For this review, use the dimensioned drawing (mm, ordinates from the lowest corner) and the shaded views. A direction names the side the tool comes from. Give positions to 0.01 mm unless a question says otherwise; leave off trailing zeros. Write each loop counter-clockwise with the first axis right and the second up, starting at its lowest first coordinate (ties: lowest second). Pieces come first, ordered by that corner, then holes. Notation, with made-up numbers: (21.25, 30.25) -> (75.25, 30.25) arc R23 ccw to (75.25, 62.25) -> close; hole circle Ø4 at (9, -34). An arc over 180 degrees is marked (long way). Return JSON: item names as keys, results as strings.
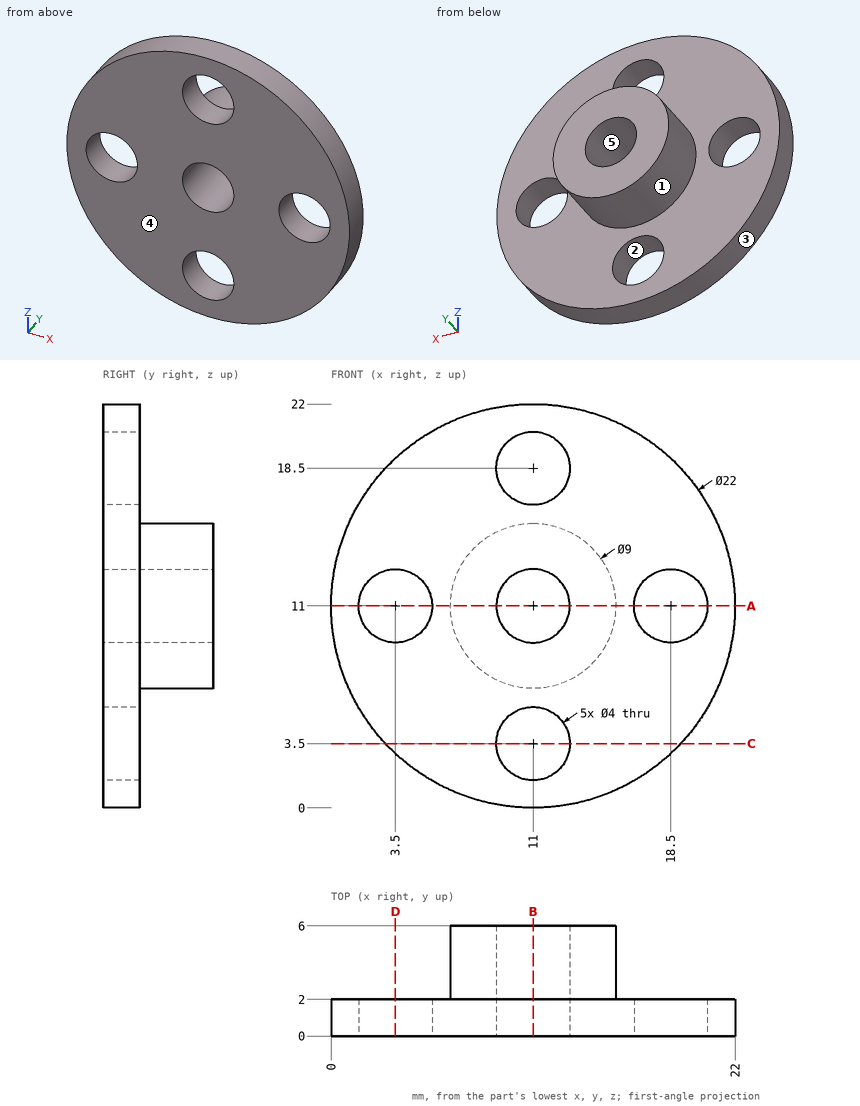
1. Add section C-C, the plane z = 3.5. State the section outline as (x, y) points.
Results found:
{"outline": "(2.95, 0) -> (9, 0) -> (9, 2) -> (2.95, 2) -> close; (13, 0) -> (19.05, 0) -> (19.05, 2) -> (13, 2) -> close"}
2. The part is to be moulded in two halves that separate along X. For the marked faces 3, 4 and 5, say which applies: +X half, -X half, draft (parallel to the pull), parting line (faces both ways), or undercut.
Results found:
{"face 3": "parting line", "face 4": "draft", "face 5": "undercut"}
3. For the marked faces 1 and 2, list the 3-axis set-ups (+Z, -Z, +X, -X, +Y, -Y) from which the entire face can be reached by the end or side of a thin tool; tool diameter is ignored.
Results found:
{"face 1": "+Y", "face 2": "+Y, -Y"}
4. Add section B-B, the plane x = 11. State the section outline as (y, z) points.
Results found:
{"outline": "(0, 0) -> (2, 0) -> (2, 1.5) -> (0, 1.5) -> close; (0, 5.5) -> (2, 5.5) -> (2, 6.5) -> (6, 6.5) -> (6, 9) -> (0, 9) -> close; (0, 13) -> (6, 13) -> (6, 15.5) -> (2, 15.5) -> (2, 16.5) -> (0, 16.5) -> close; (0, 20.5) -> (2, 20.5) -> (2, 22) -> (0, 22) -> close"}
5. Add section D-D, the plane x = 3.5. State the section outline as (y, z) points.
Results found:
{"outline": "(0, 2.95) -> (2, 2.95) -> (2, 9) -> (0, 9) -> close; (0, 13) -> (2, 13) -> (2, 19.05) -> (0, 19.05) -> close"}
6. Add section A-A, the plane z = 11. State the section outline as (x, y) points, plus the area to 3 significant figures.
Results found:
{"outline": "(0, 0) -> (1.5, 0) -> (1.5, 2) -> (0, 2) -> close; (5.5, 0) -> (9, 0) -> (9, 6) -> (6.5, 6) -> (6.5, 2) -> (5.5, 2) -> close; (13, 0) -> (16.5, 0) -> (16.5, 2) -> (15.5, 2) -> (15.5, 6) -> (13, 6) -> close; (20.5, 0) -> (22, 0) -> (22, 2) -> (20.5, 2) -> close", "area": "40.0 mm²"}
7. To check wall thickness, follow probe 1 along X at (y, z) = (1.9, 11); probe 2 along Y at (x, z) = (9.5, 1.5); probe 3 along X at (y, z) = (0.8, 18.5). State the ranges of each line that lie inside material, in increasing order.
Results found:
{"probe 1": "x = 0 to 1.5, 5.5 to 9, 13 to 16.5, 20.5 to 22", "probe 2": "y = 0 to 2", "probe 3": "x = 2.95 to 9, 13 to 19.05"}
8. For pin 1 (3.5 mm diameter, centred on x = 11, z = 11, fed in from +Y); pin 2 (3 mm diameter, centred on x = 4, z = 17, fed in from +Y), all flat-tipped, find the tip position at first contact; note any pin that passes through.
Results found:
{"pin 1": "passes through", "pin 2": "stops at y = 2"}
